Answer from the drawing. Dimensions are ordinates in mm from the lowest x, y and z of the part. A direction names the side the tool comes from. Give positions to 0.01 mm unless a question says otherwise; leave off trailing zeros. Write each loop counter-clockwise with the first axis right and the second up, starting at its lowest first coordinate (ties: lowest second). Pieces come first, ordered by that corner, then holes.
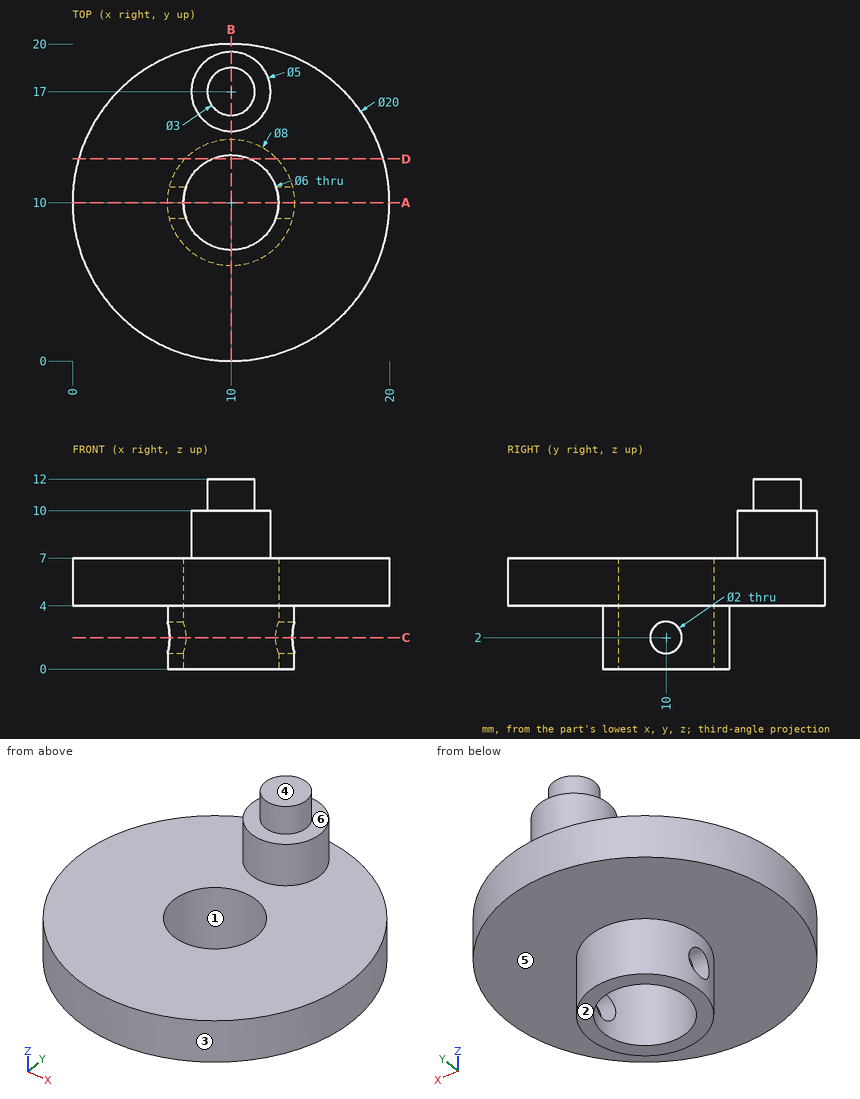
Item 1: A cutting plane is placed at D-D, the plane y = 12.75. Give the vertices of the cut face in (x, z), plus the area to 3 significant figures.
Conclusion:
outline: (0.39, 4) - (7.1, 4) - (7.1, 0) - (8.8, 0) - (8.8, 7) - (0.39, 7) - close; (11.2, 0) - (12.9, 0) - (12.9, 4) - (19.61, 4) - (19.61, 7) - (11.2, 7) - close
area: 64.1 mm2
Item 2: A cutting plane is placed at C-C, the plane z = 2. Give the vertices of the cut face in (x, y).
Conclusion:
outline: (6.13, 9) arc R4 ccw to (13.87, 9) - (12.83, 9) arc R3 cw to (7.17, 9) - close; (6.13, 11) - (7.17, 11) arc R3 cw to (12.83, 11) - (13.87, 11) arc R4 ccw to start
Item 3: Which of the six approach directions +Z, -Z, +X, -X, +Y, -Y give full straight-line access (tool end or side, diameter ignored) to the marked faces 4, 5 and 6?
Conclusion:
face 4: +Z, +X, -X, +Y, -Y
face 5: -Z
face 6: +Z
Item 4: A cutting plane is placed at B-B, the plane x = 10. Give the vertices of the cut face in (y, z).
Conclusion:
outline: (0, 4) - (6, 4) - (6, 0) - (7, 0) - (7, 7) - (0, 7) - close; (13, 0) - (14, 0) - (14, 4) - (20, 4) - (20, 7) - (19.5, 7) - (19.5, 10) - (18.5, 10) - (18.5, 12) - (15.5, 12) - (15.5, 10) - (14.5, 10) - (14.5, 7) - (13, 7) - close
Item 5: Determine the mould class of the marked faces 1, 2 and 3 for opening direction Y: pulls with the +Y half, pulls with the -Y half, needs draft (parallel to the pull), parting line crosses it, or undercut.
Conclusion:
face 1: undercut
face 2: needs draft
face 3: parting line crosses it
Item 6: Consider probe 1 along Z at (x, y) = (13.55, 10); probe 2 along Z at (x, y) = (13.25, 17); probe 3 along X at (y, z) = (12.25, 2.25). Determine where each line is inside the solid, lowest interval first.
Conclusion:
probe 1: z = 0 to 1, 3 to 7
probe 2: z = 4 to 7
probe 3: x = 6.69 to 8.02, 11.98 to 13.31
Item 7: Each of these flat-tipped pins is pushed along its axis until it touches: P1, Ø7, axis at x = 10, y = 10, coming from the +Z side; P2, Ø1, axis at x = 9.5, z = 1.5, coming from the +Y side; P3, Ø10, axis at x = 17, y = 16, coming from the +Z side; P4, Ø1.8, axis at y = 10, z = 2, coming from the +X side. Where does it stop, or does it pass through?
Conclusion:
P1: stops at z = 7
P2: stops at y = 14
P3: stops at z = 10
P4: passes through
Item 8: A cutting plane is placed at A-A, the plane y = 10. Give the vertices of the cut face in (x, z).
Conclusion:
outline: (0, 4) - (6, 4) - (6, 3) - (7, 3) - (7, 7) - (0, 7) - close; (6, 0) - (7, 0) - (7, 1) - (6, 1) - close; (13, 0) - (14, 0) - (14, 1) - (13, 1) - close; (13, 3) - (14, 3) - (14, 4) - (20, 4) - (20, 7) - (13, 7) - close
